Geometry check sheet. Reference: the model listing, model coordinates, mm. A direction names the side the tool comes from. Coordinates: 2 decimals unless noted, no trailing zeros. Write each loop counter-clockwise with the first axis right and the second up, starting at its lowest first coordinate (ties: lowest second). Pieces come first, ordered by that corner, then holes. Notation, with made-up numbers: (31, -26.5) -> (57, -26.5) arc R23 cw to (57, -6.5) -> close; hole circle Ø8 at (48.25, -29.5). An arc over 180 degrees is marked (long way). One line per question, with ' | ' between items.
from build123d import *

# Parameters (mm, degrees)
SKETCH_1_W          = 190
SKETCH_1_H          = 50
EXTRUDE_1_DEPTH     = 8
CUT_EXTRUDE_1_DEPTH = 8
CHAMFER_1_SIZE      = 5
HOLE_WIZARD_M6_1_D  = 5
FILLET_1_R          = 5


with BuildPart() as part:
    # 草图1 → 凸台-拉伸1 (new body)
    with BuildSketch(Plane.XY):
        Rectangle(SKETCH_1_W, SKETCH_1_H)
    extrude(amount=EXTRUDE_1_DEPTH)

    # 草图2 → 切除-拉伸1 (cut)
    with BuildSketch(Plane.XY.offset(8)):
        Polygon((-95, -5), (-85, 5), (-80, 5), (-80, 25), (-50, 25), (-50, 5), (50, 5), (50, 25), (80, 25), (80, 5), (85, 5), (95, -5), (95, 25), (-3.801071979, 36.264806318), (-95, 25), align=None)
    extrude(amount=-CUT_EXTRUDE_1_DEPTH, mode=Mode.SUBTRACT)

    # 倒角1
    chamfer_1_edges = [part.edges().sort_by_distance(p)[0] for p in [
        (80, 25, 4),
        (50, 25, 4),
        (-50, 25, 4),
        (-80, 25, 4),
    ]]
    chamfer(chamfer_1_edges, length=CHAMFER_1_SIZE)

    # M6 螺纹孔1 (through all)
    with Locations(Plane.XY.offset(8)):
        with Locations((-65, 13), (65, 13)):
            Hole(HOLE_WIZARD_M6_1_D / 2)

    # 圆角1
    fillet_1_edges = [part.edges().sort_by_distance(p)[0] for p in [
        (50, 5, 4),
        (-50, 5, 4),
    ]]
    fillet(fillet_1_edges, radius=FILLET_1_R)


solid = part.part
1. Cross-section at A-A on y = 13. Record the boundary of the cut face in (x, z).
Worked answers:
outline: (-80, 0) -> (-67.5, 0) -> (-67.5, 8) -> (-80, 8) -> close; (-62.5, 0) -> (-50, 0) -> (-50, 8) -> (-62.5, 8) -> close; (50, 0) -> (62.5, 0) -> (62.5, 8) -> (50, 8) -> close; (67.5, 0) -> (80, 0) -> (80, 8) -> (67.5, 8) -> close
2. Cross-section at C-C on z = 5.75. Record the boundary of the cut face in (x, y).
Worked answers:
outline: (-95, -25) -> (95, -25) -> (95, -5) -> (85, 5) -> (80, 5) -> (80, 20) -> (75, 25) -> (55, 25) -> (50, 20) -> (50, 10) arc R5 cw to (45, 5) -> (-45, 5) arc R5 cw to (-50, 10) -> (-50, 20) -> (-55, 25) -> (-75, 25) -> (-80, 20) -> (-80, 5) -> (-85, 5) -> (-95, -5) -> close; hole circle Ø5 at (-65, 13); hole circle Ø5 at (65, 13)
3. Mould release check, pull along X, two halves, no side actions. Record for faces 5 (the face through (-50, 15, 4)), 6 (the face through (48, 6, 4)), 7 (the face through (-80, 12, 4)), 8 (the face through (-1, -5, 0)): released by +X, released by -X, zero draft, split by the parting line, or undercut.
Worked answers:
face 5: undercut | face 6: undercut | face 7: released by -X | face 8: zero draft
4. Cross-section at B-B on x = -65. Record the boundary of the cut face in (y, z).
Worked answers:
outline: (-25, 0) -> (10.5, 0) -> (10.5, 8) -> (-25, 8) -> close; (15.5, 0) -> (25, 0) -> (25, 8) -> (15.5, 8) -> close
5. Cross-section at D-D on x = -21.5. Record the boundary of the cut face in (y, z).
Worked answers:
outline: (-25, 0) -> (5, 0) -> (5, 8) -> (-25, 8) -> close
6. Go/stop test with flat-tipped pins: P1, Ø2.5, axis at x = -81.5, z = 3, coming from the +Y side; P2, Ø4, axis at y = 15, z = 4, coming from the +X side; P3, Ø2, axis at y = 8.5, z = 6, coming from the -X side. Record where each tip stops, or that it passes through.
Worked answers:
P1: y = 5 | P2: x = 80 | P3: x = -80
7. Tool access check on faces 1 (the face through (-65, 25, 4)), 2 (the face through (50, 15, 4)), 3 (the face through (-83, 5, 4)), 4 (the face through (82, 5, 4)). Record the directions out of +Z, -Z, +X, -X, +Y, -Y that give a thin tool (end or side, any length) a straight path to the whole face; none if there is none.
Worked answers:
face 1: +Z, -Z, +X, -X, +Y | face 2: +Z, -Z, +Y | face 3: +Z, -Z, -X, +Y | face 4: +Z, -Z, +X, +Y
8. Material ranges on line 1 (Y direction, x = 65, z = 4); line 2 (X direction, y = 15, z = 7.5); line 3 (Y direction, x = -25, z = 2.25), recorded low to high. Write a range as from..to.
Worked answers:
line 1: -25..10.5, 15.5..25 | line 2: -80..-66.5, -63.5..-50, 50..63.5, 66.5..80 | line 3: -25..5
